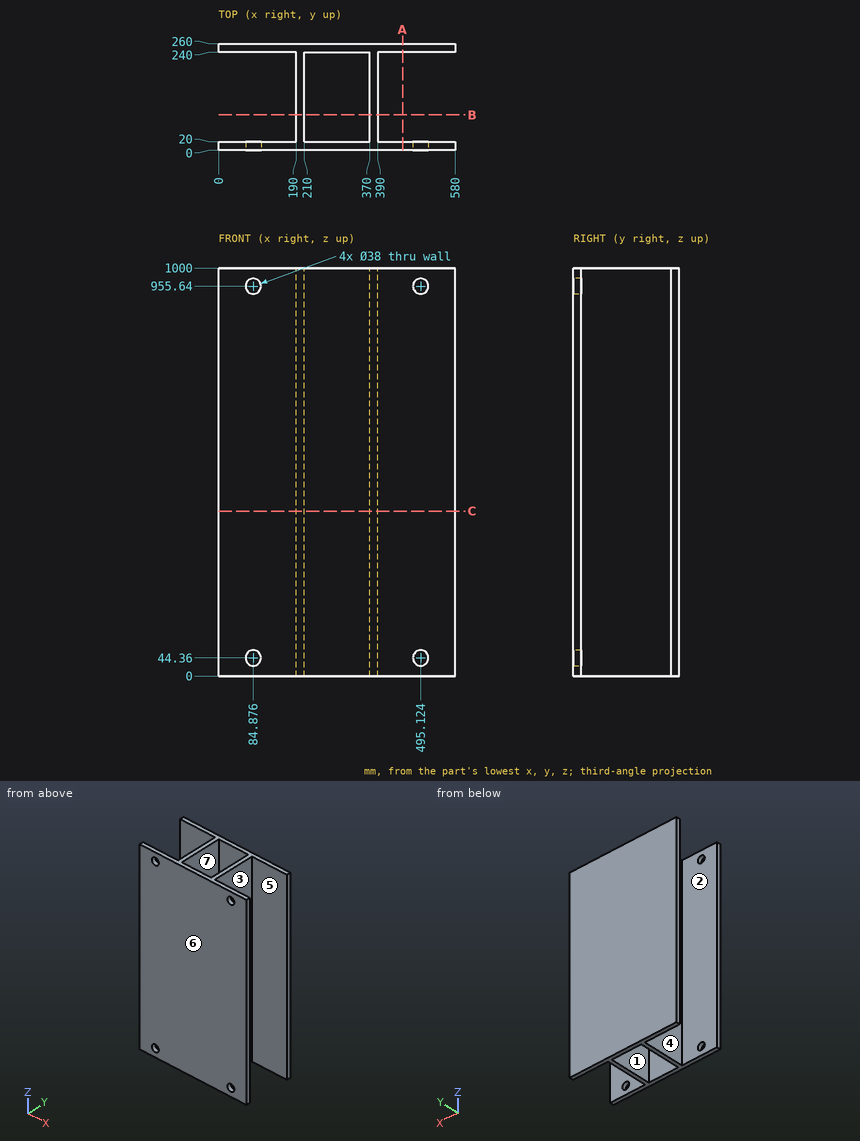
Check sheet for the drawn part. Datum: minimum x, y, z corner. Units: mm. A direction names the side the tool comes from. Give positions to 0.01 mm unless a question says otherwise; leave off trailing zeros. Order: outer loops, then holes, each group sorted by start corner. A loop starts at its lowest first (then second) coordinate and runs counter-clockwise, first axis right, second up. Notation, with made-up numbers: (-27.5, 76) -> (14.5, 76) arc R22 cw to (14.5, 89) -> close; hole circle Ø3 at (45.5, 79). An arc over 180 degrees is marked (long way). Answer as CSV lines item,"result".
Q1. Depth check by flat-ended pin: pin 1 (1 mm diameter, centred on y = 105, z = 707.5, fed in from +X); pin 2 (6 mm diameter, centred on y = 85, z = 588, fed in from -X). Enter the tip coordinate at first touch or a pass-through.
Solutions:
pin 1,"stops at x = 390"
pin 2,"stops at x = 190"
Q2. Sectioned sample at B-B on y = 86. Record the cut outline in (x, z), plus the area to 3 significant figures.
Solutions:
outline,"(190, 0) -> (210, 0) -> (210, 1000) -> (190, 1000) -> close; (370, 0) -> (390, 0) -> (390, 1000) -> (370, 1000) -> close"
area,"40,000 mm²"
Q3. Sectioned sample at C-C on z = 404. Record the cut outline in (x, y).
Solutions:
outline,"(0, 0) -> (580, 0) -> (580, 20) -> (390, 20) -> (390, 240) -> (580, 240) -> (580, 260) -> (0, 260) -> (0, 240) -> (190, 240) -> (190, 20) -> (0, 20) -> close; hole (210, 20) -> (370, 20) -> (370, 240) -> (210, 240) -> close"
Q4. Access from +Z, -Z, +X, -X, +Y, -Y to the whole of each face (thin tool, end or side, straight path). Record for the marked faces 4, 5, 6 and 7.
Solutions:
face 4,"+Z, -Z, -X"
face 5,"+Z, -Z, +X"
face 6,"+Z, -Z, +X, -X, -Y"
face 7,"+Z, -Z"
Q5. Release check for a two-part mould opening along X. For the marked faces 1, 2 and 3 record: +X half, -X half, draft (parallel to the pull), parting line (faces both ways), or undercut.
Solutions:
face 1,"undercut"
face 2,"draft"
face 3,"+X half"
Q6. Sectioned sample at A-A on x = 451. Record the cut outline in (y, z), plus the area to 3 significant figures.
Solutions:
outline,"(0, 0) -> (20, 0) -> (20, 1000) -> (0, 1000) -> close; (240, 0) -> (260, 0) -> (260, 1000) -> (240, 1000) -> close"
area,"40,000 mm²"
Q7. Scan lines: probe 1 along X at (y, z) = (120, 726); probe 2 along Y at (x, z) = (249, 958). Record each from-to range of solid material in increasing order.
Solutions:
probe 1,"x = 190 to 210, 370 to 390"
probe 2,"y = 0 to 20, 240 to 260"
